Verification items for the finished model (mm, model axes). A direction names the side the tool comes from. Round coordinates to 2 decimals unless told otherwise and drop trailing zeros. Loops run counter-clockwise (first coordinate to the right, second up) from the corner with the lowest first, then second, coordinate; pieces in that order, holes last. Notation, with made-up numbers: M 73,46 L 90,46 A3 cw 90,50 Z; hole C 60,37.25 d10. An arc over 180 degrees is marked long. One line per item, written item: value.
from build123d import *

# Parameters (mm, degrees)
SKETCH_1_W          = 180
SKETCH_1_H          = 182
EXTRUDE_1_DEPTH     = 7
SKETCH_2_W          = 60
SKETCH_2_H          = 64
SKETCH_2_H_2        = 22
CUT_EXTRUDE_1_DEPTH = 1.5
CUT_EXTRUDE_2_DEPTH = 1.5
CUT_EXTRUDE_3_REACH = 130.752
SKETCH_4_W          = 150
SKETCH_4_H          = 86
FILLET_1_R          = 3
CUT_EXTRUDE_4_REACH = 205.158
SKETCH_6_R          = 3.5
SKETCH_7_W          = 15
SKETCH_7_H          = 182
CUT_EXTRUDE_5_DEPTH = 1.5


with BuildPart() as part:
    # 草图1 → 凸台-拉伸1 (new, symmetric)
    with BuildSketch(Plane.XY):
        Rectangle(SKETCH_1_W, SKETCH_1_H)
    extrude(amount=EXTRUDE_1_DEPTH, both=True)

    # 草图2 → 切除-拉伸1 (cut)
    with BuildSketch(Plane(origin=(0, 0, -7), x_dir=(-1, 0, 0), z_dir=(0, 0, -1))):
        with Locations((0, 59)):
            Rectangle(SKETCH_2_W, SKETCH_2_H)
        with Locations((0, -80)):
            Rectangle(SKETCH_2_W, SKETCH_2_H_2)
    extrude(amount=-CUT_EXTRUDE_1_DEPTH, mode=Mode.SUBTRACT)

    # 草图3 → 切除-拉伸2 (cut)
    with BuildSketch(Plane(origin=(0, 0, -7), x_dir=(-1, 0, 0), z_dir=(0, 0, -1))):
        with BuildLine():
            Line((30, 27), (32, 27))
            ThreePointArc((32, 27), (37, 32), (32, 37))
            Line((32, 37), (30, 37))
            Line((30, 37), (30, 27))
        make_face()
        with BuildLine():
            Line((-30, 37), (-30, 27))
            Line((-30, 27), (-32, 27))
            ThreePointArc((-32, 27), (-37, 32), (-32, 37))
            Line((-32, 37), (-30, 37))
        make_face()
        with BuildLine():
            Line((30, -69), (32, -69))
            ThreePointArc((32, -69), (37, -74), (32, -79))
            Line((32, -79), (30, -79))
            Line((30, -79), (30, -69))
        make_face()
        with BuildLine():
            Line((-30, -79), (-30, -69))
            Line((-30, -69), (-32, -69))
            ThreePointArc((-32, -69), (-37, -74), (-32, -79))
            Line((-32, -79), (-30, -79))
        make_face()
    extrude(amount=-CUT_EXTRUDE_2_DEPTH, mode=Mode.SUBTRACT)

    # 草图4 → 切除-拉伸3 (cut, up to next)
    with BuildSketch(Plane(origin=(0, 0, -7), x_dir=(-1, 0, 0), z_dir=(0, 0, -1)), mode=Mode.PRIVATE) as cut_extrude_3_sk1:
        with Locations((0, -21)):
            Rectangle(SKETCH_4_W, SKETCH_4_H)
    cut_extrude_3_tool1 = extrude(cut_extrude_3_sk1.sketch, amount=-CUT_EXTRUDE_3_REACH, mode=Mode.PRIVATE) & part.part
    add(cut_extrude_3_tool1.solids().sort_by_distance((0, -21, -7))[0], mode=Mode.SUBTRACT)

    # 圆角1
    fillet_1_edges = [part.edges().sort_by_distance(p)[0] for p in [
        (-75, 22, 0),
        (-75, -64, 0),
        (75, -64, 0),
        (75, 22, 0),
    ]]
    fillet(fillet_1_edges, radius=FILLET_1_R)

    # 草图6 → 切除-拉伸4 (cut, up to next)
    with BuildSketch(Plane.XZ.offset(91), mode=Mode.PRIVATE) as cut_extrude_4_sk1:
        with Locations(Location((-28, 0, 0), (0, 0, 270))):
            Circle(SKETCH_6_R)
    cut_extrude_4_tool1 = extrude(cut_extrude_4_sk1.sketch, amount=-CUT_EXTRUDE_4_REACH, mode=Mode.PRIVATE) & part.part
    # 草图6 → 切除-拉伸4 (cut, up to next)
    with BuildSketch(Plane.XZ.offset(91), mode=Mode.PRIVATE) as cut_extrude_4_sk2:
        with Locations(Location((28, 0, 0), (0, 0, 270))):
            Circle(SKETCH_6_R)
    cut_extrude_4_tool2 = extrude(cut_extrude_4_sk2.sketch, amount=-CUT_EXTRUDE_4_REACH, mode=Mode.PRIVATE) & part.part
    # 草图6 → 切除-拉伸4 (cut, up to next)
    with BuildSketch(Plane.XZ.offset(91), mode=Mode.PRIVATE) as cut_extrude_4_sk3:
        with Locations(Location((-5, 0, 0), (0, 0, 270))):
            Circle(SKETCH_6_R)
    cut_extrude_4_tool3 = extrude(cut_extrude_4_sk3.sketch, amount=-CUT_EXTRUDE_4_REACH, mode=Mode.PRIVATE) & part.part
    # 草图6 → 切除-拉伸4 (cut, up to next)
    with BuildSketch(Plane.XZ.offset(91), mode=Mode.PRIVATE) as cut_extrude_4_sk4:
        with Locations(Location((5, 0, 0), (0, 0, 270))):
            Circle(SKETCH_6_R)
    cut_extrude_4_tool4 = extrude(cut_extrude_4_sk4.sketch, amount=-CUT_EXTRUDE_4_REACH, mode=Mode.PRIVATE) & part.part
    add(cut_extrude_4_tool1.solids().sort_by_distance((-28, -91, 0))[0], mode=Mode.SUBTRACT)
    add(cut_extrude_4_tool2.solids().sort_by_distance((28, -91, 0))[0], mode=Mode.SUBTRACT)
    add(cut_extrude_4_tool3.solids().sort_by_distance((-5, -91, 0))[0], mode=Mode.SUBTRACT)
    add(cut_extrude_4_tool4.solids().sort_by_distance((5, -91, 0))[0], mode=Mode.SUBTRACT)

    # 草图7 → 切除-拉伸5 (cut)
    with BuildSketch(Plane.XY.offset(7)):
        with Locations((-82.5, 0)):
            Rectangle(SKETCH_7_W, SKETCH_7_H)
        with Locations((82.5, 0)):
            Rectangle(SKETCH_7_W, SKETCH_7_H)
    extrude(amount=-CUT_EXTRUDE_5_DEPTH, mode=Mode.SUBTRACT)


solid = part.part
(1) Depth check by flat-ended pin: pin 1 Ø17.5 at (x, y) = (-15.5, -76.5) entering from -Z; pin 2 Ø4 at (x, z) = (-5, 0) entering from -Y; pin 3 Ø1.2 at (y, z) = (-80.5, 6.5) entering from +X. Enter the tip coordinate at first touch or a pass-through.
Completed:
pin 1: stops at z = -7
pin 2: stops at y = 22
pin 3: stops at x = 75
(2) Sectioned sample at B-B on y = -32. Enter the section's corners in (x, z), and give its area (3 significant figures).
Completed:
outline: M -90,-7 L -75,-7 L -75,5.5 L -90,5.5 Z; M 75,-7 L 90,-7 L 90,5.5 L 75,5.5 Z
area: 375 mm^2
(3) Mould release check, pull along X, two halves, no side actions. Record for faces 1 (the face through (-90, -1, -1)), 2 (the face through (75, -22, -1)), 3 (the face through (82, 1, 5.5)), 4 (the face through (90, -1, -1)): +X half, -X half, draft (parallel to the pull), parting line (faces both ways), or undercut.
Completed:
face 1: -X half
face 2: undercut
face 3: draft
face 4: +X half
(4) Thickness scan on L1, parallel to X at y = -79, z = 0; L2, parallel to Y at x = -33, z = -4.5; L3, parallel to X at y = -4, z = 2.5. Record the ranges inside material, lowest first. Write a range as from..to.
Completed:
L1: x = -90..-31.5, -24.5..-8.5, -1.5..1.5, 8.5..24.5, 31.5..90
L2: y = -91..-64, 22..91
L3: x = -90..-75, 75..90
(5) Tool access check on faces 5 (the face through (1, 22, 0)), 6 (the face through (1.583, -77.689, 0.759)), 7 (the face through (37, 32, -6)). Record the directions out of +Z, -Z, +X, -X, +Y, -Y that give a thin tool (end or side, any length) a straight path to the whole face; none if there is none.
Completed:
face 5: +Z, -Z
face 6: -Y
face 7: -Z
(6) Sectioned sample at D-D on x = 45. Enter the section's corners in (y, z), and give its area (3 significant figures).
Completed:
outline: M -91,-7 L -64,-7 L -64,7 L -91,7 Z; M 22,-7 L 91,-7 L 91,7 L 22,7 Z
area: 1,340 mm^2
(7) Sectioned sample at C-C on z = 0. Enter the section's corners in (x, y).
Completed:
outline: M -90,-91 L -31.5,-91 L -31.5,-64 L -72,-64 A3 cw -75,-61 L -75,19 A3 cw -72,22 L 72,22 A3 cw 75,19 L 75,-61 A3 cw 72,-64 L 31.5,-64 L 31.5,-91 L 90,-91 L 90,91 L -90,91 Z; M -24.5,-91 L -8.5,-91 L -8.5,-64 L -24.5,-64 Z; M -1.5,-91 L 1.5,-91 L 1.5,-64 L -1.5,-64 Z; M 8.5,-91 L 24.5,-91 L 24.5,-64 L 8.5,-64 Z
(8) Sectioned sample at A-A on x = 5. Enter the section's corners in (y, z), and give its area (3 significant figures).
Completed:
outline: M -91,-5.5 L -69,-5.5 L -69,-7 L -64,-7 L -64,-3.5 L -91,-3.5 Z; M -91,3.5 L -64,3.5 L -64,7 L -91,7 Z; M 22,-7 L 27,-7 L 27,-5.5 L 91,-5.5 L 91,7 L 22,7 Z
area: 1,030 mm^2
